Geometry: final body of the model. Coordinates: model frame, mm. A direction names the side the tool comes from. Coordinates: 2 decimals unless noted, no trailing zeros. Write each loop counter-clockwise with the first axis right and the second up, starting at its lowest first coordinate (ties: lowest second). Pieces come first, ordered by that corner, then holes. Notation, with made-up numbers: (21, -20.5) - (26, -20.5) arc R16 cw to (26, -4.5) - close; hole circle Ø8 at (3.5, 44.5). An arc over 180 degrees is marked (long way). Answer as a JSON object with one key per item and string values. Group by question number.
Item 1: Section A-A on x = 0. Return loops of the section in (y, z), and give its area (4 significant figures).
Item 2: Line query: line 1 along X through (y, z) = (6.5, 0); line 2 along Y through (x, z) = (-17, -3); line 3 along X through (y, z) = (12, -4). Output: solid intervals per line, ascending. Write a range as from..to.
Item 3: Section D-D on z = -14.5. Return loops of the section in (x, y), and give its area (3 significant figures).
Item 4: Section B-B on z = 0. Return loops of the section in (x, y), and give its area (4 significant figures).
Item 5: Set-up query: faces 1 (the flat face through (-16.4, 10, -2.9)), 2 (the flat face through (-12.3, 13.5, 2.5)). Return all of +Z, -Z, +X, -X, +Y, -Y with unobstructed straight access to the full face (end or side cutting, diameter ignored); none if empty.
Item 6: Mould query, pull axis Z, two halves, no side actions, for faces 3 (the cylindrical face through (-4.956, 11.774, -15.738)), 4 (the flat face through (13, 0, -5)), 5 (the cylindrical face through (-6.586, 7.416, -10.329)). Classes: pulls with the +Z half, pulls with the -Z half, needs draft (parallel to the pull), parting line crosses it, or undercut.
Item 7: First-contact query: pin 1 Ø1.5 at (y, z) = (9.5, -1) entering from -X; pin 2 Ø1 at (x, y) = (1, 1.5) entering from -Z; pin 3 Ø1 at (y, z) = (8.5, -7.5) entering from -X (3 decimals). Flat tips, straight axial feed; report the tip coordinate or a pass-through.
Item 8: Section C-C on y = 2. Return loops of the section in (x, z), and give its area (3 significant figures).
```python
from build123d import *

# Parameters (mm, degrees)
G3_4_TAPPED_HOLE1_D     = 24.5
G3_4_TAPPED_HOLE1_DEPTH = 58.32
G3_4_TAPPED_HOLE1_TIP   = 7.360542583
CHAMFER1_SIZE           = 1.5


with BuildPart() as part:
    # Sketch1 → Revolve1 (revolve)
    with BuildSketch(Plane.XY, mode=Mode.PRIVATE) as revolve1_sk:
        Polygon((0, 0), (20, 0), (20, 10), (16.5, 10), (16.5, 13.5), (0, 13.5), align=None)
    revolve(revolve1_sk.sketch.rotate(Axis((0, 0, 0), (0, 1, 0)), 90), axis=Axis((0, 0, 0), (0, 1, 0)))

    # G3/4 Tapped Hole1
    with Locations(Plane(origin=(0, 13.5, 0), x_dir=(1, 0, 0), z_dir=(0, 1, 0))):
        with Locations((0, 0)):
            Hole(G3_4_TAPPED_HOLE1_D / 2, depth=G3_4_TAPPED_HOLE1_DEPTH)
            with Locations((0, 0, -(G3_4_TAPPED_HOLE1_DEPTH + G3_4_TAPPED_HOLE1_TIP / 2))):  # 118° drill point
                Cone(0, G3_4_TAPPED_HOLE1_D / 2, G3_4_TAPPED_HOLE1_TIP, mode=Mode.SUBTRACT)

    # Chamfer1
    chamfer1_edges = [part.edges().sort_by_distance(p)[0] for p in [
        (12.25, 0, 0),
    ]]
    chamfer(chamfer1_edges, length=CHAMFER1_SIZE)


solid = part.part
```
Checks:
{
 "1": {"outline": "(0, -20) - (10, -20) - (10, -16.5) - (13.5, -16.5) - (13.5, -12.25) - (1.5, -12.25) - (0, -13.75) - close; (0, 13.75) - (1.5, 12.25) - (13.5, 12.25) - (13.5, 16.5) - (10, 16.5) - (10, 20) - (0, 20) - close", "area": "182.5 mm^2"},
 "2": {"line 1": "-20..-12.25, 12.25..20", "line 2": "0..10", "line 3": "-16.01..-11.58, 11.58..16.01"},
 "3": {"outline": "(-13.77, 0) - (13.77, 0) - (13.77, 10) - (7.87, 10) - (7.87, 13.5) - (-7.87, 13.5) - (-7.87, 10) - (-13.77, 10) - close", "area": "331 mm^2"},
 "4": {"outline": "(-20, 0) - (-13.75, 0) - (-12.25, 1.5) - (-12.25, 13.5) - (-16.5, 13.5) - (-16.5, 10) - (-20, 10) - close; (12.25, 1.5) - (13.75, 0) - (20, 0) - (20, 10) - (16.5, 10) - (16.5, 13.5) - (12.25, 13.5) - close", "area": "182.5 mm^2"},
 "5": {"face 1": "+Y", "face 2": "+Z, -Z, +X, -X, +Y"},
 "6": {"face 3": "parting line crosses it", "face 4": "needs draft", "face 5": "undercut"},
 "7": {"pin 1": "x = -20", "pin 2": "z = -19.99", "pin 3": "x = -18.735"},
 "8": {"outline": "circle Ø40 at (0, 0); hole circle Ø24.5 at (0, 0)", "area": "785 mm^2"}
}
